Input: dimensioned drawing with shaded views. Units: mm. Origin: part minimum x, y, z. A direction names the side the tool comes from. Give positions to 0.01 mm unless a question says otherwise; leave off trailing zeros. Write each loop counter-clockwise with the first axis right and the second up, starting at its lowest first coordinate (ties: lowest second). Pieces come first, ordered by that corner, then holes. Notation, with made-up numbers: (13.25, 9.25) -> (34.25, 9.25) arc R17 ccw to (34.25, 21.25) -> close; hole circle Ø1 at (73.5, 70.5). An arc over 180 degrees is marked (long way). Answer as a JSON object with one key per item and string values.
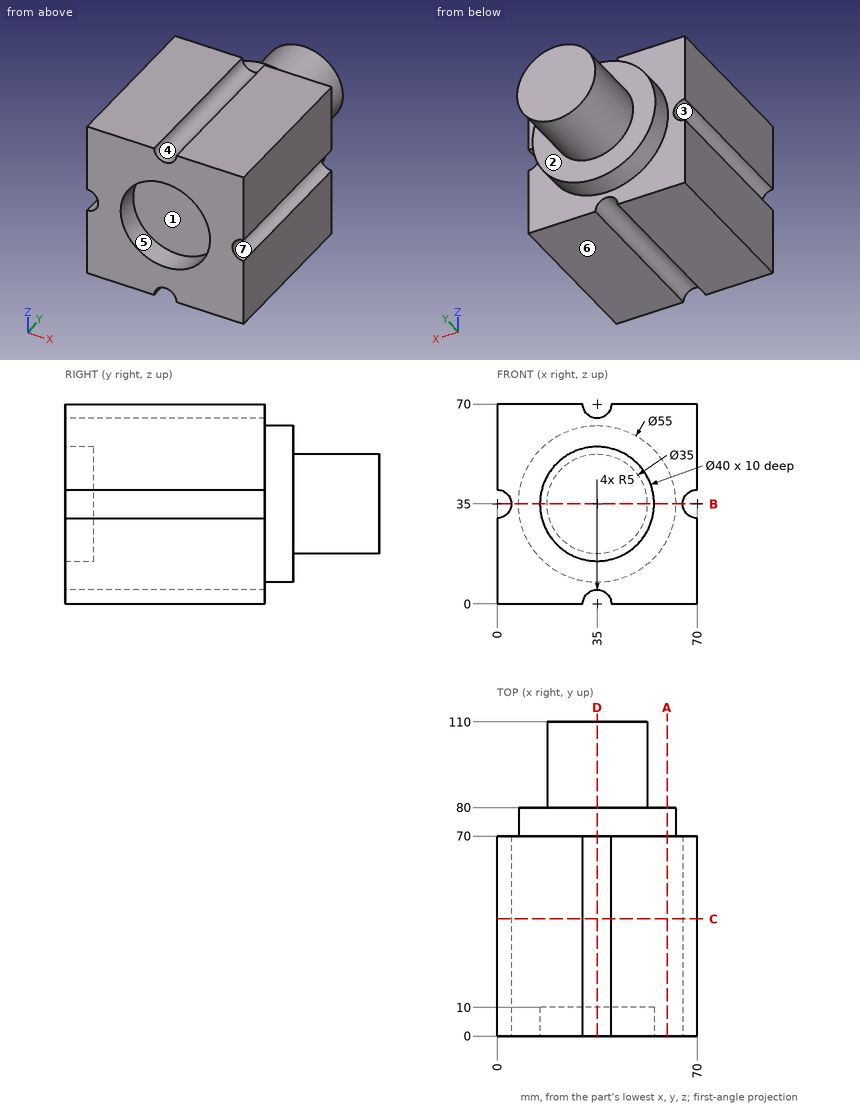
Q1. Material intervals for L1, parallel to X at y = 2.5, z = 35; L2, parallel to Y at x = 18, z = 28.5; L3, parallel to Y at x = 13.5, z = 8.5, sorted ascending. Write a range as from..to.
Values:
{"L1": "5..15, 55..65", "L2": "10..80", "L3": "0..70"}
Q2. Mould query, pull axis X, two halves, no side actions, for the marked faces 4, 5, 6 and 7. Classes: pulls with the +X half, pulls with the -X half, needs draft (parallel to the pull), parting line crosses it, or undercut.
Values:
{"face 4": "undercut", "face 5": "undercut", "face 6": "needs draft", "face 7": "pulls with the +X half"}
Q3. Cut plane A-A (x = 59.5). Return the cut outline in (y, z), and give its area (3 significant figures).
Values:
{"outline": "(0, 0) -> (70, 0) -> (70, 22.51) -> (80, 22.51) -> (80, 47.49) -> (70, 47.49) -> (70, 70) -> (0, 70) -> close", "area": "5,150 mm²"}
Q4. Set-up query: the marked faces 1, 2 and 3. Return all of +Z, -Z, +X, -X, +Y, -Y with unobstructed straight access to the full face (end or side cutting, diameter ignored); none if empty.
Values:
{"face 1": "-Y", "face 2": "+Y", "face 3": "-X, +Y, -Y"}
Q5. First-contact query: P1, Ø2, axis at x = 41, z = 33, coming from the -Y side; P2, Ø2, axis at x = 24, y = 73.5, coming from the -Z side; P3, Ø6, axis at x = 24.5, z = 59, coming from the -Y side. Flat tips, straight axial feed; report the tip coordinate or a pass-through.
Values:
{"P1": "y = 10", "P2": "z = 9.38", "P3": "y = 0"}
Q6. Cut plane C-C (y = 41). Return the cut outline in (x, z), and give its area (3 significant figures).
Values:
{"outline": "(0, 0) -> (30, 0) arc R5 cw to (40, 0) -> (70, 0) -> (70, 30) arc R5 cw to (70, 40) -> (70, 70) -> (40, 70) arc R5 cw to (30, 70) -> (0, 70) -> (0, 40) arc R5 cw to (0, 30) -> close", "area": "4,740 mm²"}
Q7. Cut plane D-D (x = 35). Return the cut outline in (y, z), and give its area (3 significant figures).
Values:
{"outline": "(0, 5) -> (70, 5) -> (70, 7.5) -> (80, 7.5) -> (80, 17.5) -> (110, 17.5) -> (110, 52.5) -> (80, 52.5) -> (80, 62.5) -> (70, 62.5) -> (70, 65) -> (0, 65) -> (0, 55) -> (10, 55) -> (10, 15) -> (0, 15) -> close", "area": "5,400 mm²"}
Q8. Cut plane B-B (z = 35). Return the cut outline in (x, y).
Values:
{"outline": "(5, 0) -> (15, 0) -> (15, 10) -> (55, 10) -> (55, 0) -> (65, 0) -> (65, 70) -> (62.5, 70) -> (62.5, 80) -> (52.5, 80) -> (52.5, 110) -> (17.5, 110) -> (17.5, 80) -> (7.5, 80) -> (7.5, 70) -> (5, 70) -> close"}
